Read the model definition and answer for the solid it produces. Units are mm, in the model's axes. A direction names the side the tool comes from. Coordinates: 2 decimals unless noted, no trailing zeros. Loops run counter-clockwise (first coordinate to the right, second up) from the corner with the lowest first, then second, coordinate; pieces in that order, holes last. Notation, with made-up numbers: M -13,22 L 23,22 A29 cw 23,50 Z; hole C -16,-19.75 d10. An arc over 180 degrees is marked long. Put each result on its own line as item: value.
from build123d import *

# Parameters (mm, degrees)
SKETCH_1_R           = 42.5
EXTRUDE_1_DEPTH      = 460
SKETCH_2_R           = 77.5
EXTRUDE_2_DEPTH      = 50
SKETCH_3_R           = 75.00000000000003
SKETCH_3_R_2         = 32.499999999999964
EXTRUDE_3_DEPTH      = 34
EXTRUDE_4_REACH      = 523.644
EXTRUDE_4_END_RADIUS = 75.00000000000003
SKETCH_4_R           = 25
FILLET_1_R           = 10


with BuildPart() as part:
    # Sketch 1 → Extrude 1 (new body)
    with BuildSketch(Plane.XY):
        Circle(SKETCH_1_R)
    extrude(amount=EXTRUDE_1_DEPTH)

    # Sketch 2 → Extrude 2 (add)
    with BuildSketch(Plane(origin=(0, 0, 0), x_dir=(-1, 0, 0), z_dir=(0, 0, -1))):
        Circle(SKETCH_2_R)
    extrude(amount=EXTRUDE_2_DEPTH)



with BuildPart() as body_2:
    # Sketch 3 → Extrude 3 (new, symmetric)
    with BuildSketch(Plane(origin=(0, 0, 0), x_dir=(0, 0, -1), z_dir=(1, 0, 0))):
        with Locations((-560, 0)):
            Circle(SKETCH_3_R)
        with Locations((-560, 0)):
            Circle(SKETCH_3_R_2, mode=Mode.SUBTRACT)
    extrude(amount=EXTRUDE_3_DEPTH, both=True)


with BuildPart() as part_1:
    add(part.part)

    add(body_2.part)  # Extrude 4 merges body 2
    # Extrude 4: up to this cylinder (the profile starts outside it)
    extrude_4_end = Plane(origin=(0, 0, 560), z_dir=(-1, 0, 0)) * Cylinder(EXTRUDE_4_END_RADIUS, 1198.288, mode=Mode.PRIVATE)
    # Sketch 4 → Extrude 4 (add, up to the surface)
    with BuildSketch(Plane.XY.offset(460), mode=Mode.PRIVATE) as extrude_4_sk1:
        with Locations(Location((0, 0, 0), (0, 0, 180))):
            Circle(SKETCH_4_R)
    extrude_4_tool1 = extrude(extrude_4_sk1.sketch, amount=EXTRUDE_4_REACH, mode=Mode.PRIVATE) - extrude_4_end
    add(extrude_4_tool1.solids().sort_by_distance((0, 0, 460))[0])

    # Fillet 1
    fillet_1_edges = [part_1.edges().sort_by_distance(p)[0] for p in [
        (-34, 9.18e-15, 635),
        (34, 9.18e-15, 635),
    ]]
    fillet(fillet_1_edges, radius=FILLET_1_R)


solid = part_1.part
1) Straight lines are drawn through the part: line 1 (Y direction, x = -17, z = 560); line 2 (Z direction, x = -15.5, y = -3); line 3 (Z direction, x = -32.5, y = -7). For each, find the intervals that lie inside material, in ascending order. Write a range as [from, to].
Answer list:
line 1: y = [-75, -32.5], [32.5, 75]
line 2: z = [-50, 527.64], [592.36, 634.94]
line 3: z = [-50, 460], [490.08, 528.26], [591.74, 629.92]
2) Find section D-D, the plane x = 51.5. Write down the section's boundary in (y, z), plus the area to 3 significant figures.
Answer list:
outline: M -57.91,-50 L 57.91,-50 L 57.91,0 L -57.91,0 Z
area: 5,790 mm^2
3) Which of the six approach directions +Z, -Z, +X, -X, +Y, -Y give full straight-line access (tool end or side, diameter ignored) to faces 5 (the flat face through (-33, -33, 0)), 6 (the cylindrical face through (-0.48, 1.43, 592.47)), 7 (the flat face through (-34, 30, 546))?
Answer list:
face 5: none
face 6: +X, -X
face 7: +Z, -X, +Y, -Y
4) Given pin 1 Ø8 at (x, z) = (-5.5, 501.5) entering from +Y; pin 2 Ø6 at (y, z) = (6, 324.5) entering from +X; pin 3 Ø1 at (x, z) = (0.5, 75.5) entering from -Y, each flat-ended and moving along its own axis, determine where each tip first touches the part or whether it passes through.
Answer list:
pin 1: stops at y = 51.52
pin 2: stops at x = 42.39
pin 3: stops at y = -42.5
5) Find section C-C, the plane z = 201.5. Write down the section's boundary in (x, y), plus the area to 3 significant figures.
Answer list:
outline: C 0,0 d85
area: 5,670 mm^2
6) Find section A-A, the plane z = 560. Write down the section's boundary in (x, y).
Answer list:
outline: M -34,-65 A10 ccw -24,-75 L 24,-75 A10 ccw 34,-65 L 34,-32.5 L -34,-32.5 Z; M -34,32.5 L 34,32.5 L 34,65 A10 ccw 24,75 L -24,75 A10 ccw -34,65 Z
7) Find section B-B, the plane x = 0. Write down the section's boundary in (y, z).
Answer list:
outline: M -77.5,-50 L 77.5,-50 L 77.5,0 L 42.5,0 L 42.5,460 L 25,460 L 25,489.29 A75 ccw long -25,489.29 L -25,460 L -42.5,460 L -42.5,0 L -77.5,0 Z; hole C 0,560 d65
8) Determine the mould class of faces 1 (the flat face through (1, 1, -50)), 2 (the flat face through (34, 30, 546)), 3 (the cylindrical face through (-23.846, -7.509, 474.44)), 4 (the cylindrical face through (0.34, 3.2, 634.93)) for opening direction Z: released by +Z, released by -Z, zero draft, split by the parting line, or undercut.
Answer list:
face 1: released by -Z
face 2: zero draft
face 3: undercut
face 4: undercut
